```python
from build123d import *

# Parameters (mm, degrees)
SKETCH1_W                                           = 570
SKETCH1_H                                           = 160
BOSS_EXTRUDE1_DEPTH                                 = 12
SKETCH2_W                                           = 24
SKETCH2_H                                           = 246.506816481
SKETCH2_W_2                                         = 20
SKETCH2_H_2                                         = 260.473208351
CUT_EXTRUDE1_DEPTH                                  = 2
SKETCH3_W                                           = 431
SKETCH3_H                                           = 32
CUT_EXTRUDE2_DEPTH                                  = 2
SKETCH4_W                                           = 12
SKETCH4_H                                           = 67
CUT_EXTRUDE3_DEPTH                                  = 297.258333216
M5_TAPPED_HOLE1_D                                   = 4.2
FILLET1_R                                           = 5
FILLET2_R                                           = 5
CHAMFER1_SIZE                                       = 2
CBORE_FOR_M5_HEX_SOCKET_HEAD_CAP_SCREW1_D           = 5.5
CBORE_FOR_M5_HEX_SOCKET_HEAD_CAP_SCREW1_CBORE_D     = 10
CBORE_FOR_M5_HEX_SOCKET_HEAD_CAP_SCREW1_CBORE_DEPTH = 5.4
SKETCH13_R                                          = 8
CUT_EXTRUDE4_DEPTH                                  = 18
SKETCH14_R                                          = 2.5
CUT_EXTRUDE5_DEPTH                                  = 12
SKETCH15_R                                          = 8
CUT_EXTRUDE6_DEPTH                                  = 12


with BuildPart() as part:
    # Sketch1 → Boss-Extrude1 (new body)
    with BuildSketch(Plane.XY):
        Rectangle(SKETCH1_W, SKETCH1_H)
    extrude(amount=BOSS_EXTRUDE1_DEPTH)

    # Sketch2 → Cut-Extrude1 (cut)
    with BuildSketch(Plane.XY.offset(12)):
        with Locations((-200, -10.474793902)):
            Rectangle(SKETCH2_W, SKETCH2_H)
        with Locations((253, -9.078154715)):
            Rectangle(SKETCH2_W_2, SKETCH2_H_2)
    extrude(amount=-CUT_EXTRUDE1_DEPTH, mode=Mode.SUBTRACT)

    # Sketch3 → Cut-Extrude2 (cut)
    with BuildSketch(Plane.XY.offset(12)):
        with Locations((27.5, 64)):
            Rectangle(SKETCH3_W, SKETCH3_H)
        with Locations((27.5, -64)):
            Rectangle(SKETCH3_W, SKETCH3_H)
    extrude(amount=-CUT_EXTRUDE2_DEPTH, mode=Mode.SUBTRACT)

    # Sketch4 → Cut-Extrude3 (cut, through all)
    with BuildSketch(Plane.XY.offset(12)):
        with Locations((-279, 0)):
            Rectangle(SKETCH4_W, SKETCH4_H)
    extrude(amount=-CUT_EXTRUDE3_DEPTH, mode=Mode.SUBTRACT)

    # M5 Tapped Hole1 (through all)
    with Locations(Plane.XY.offset(10)):
        with Locations((227.5, -59), (107.5, -59), (-172.5, -59), (-52.5, -59), (-172.5, 59), (-52.5, 59), (107.5, 59), (227.5, 59)):
            Hole(M5_TAPPED_HOLE1_D / 2)

    # Fillet1
    fillet1_edges = [part.edges().sort_by_distance(p)[0] for p in [
        (-188, 48, 11),
        (243, 48, 11),
        (-188, -48, 11),
        (243, -48, 11),
    ]]
    fillet(fillet1_edges, radius=FILLET1_R)

    # Fillet2
    fillet2_edges = [part.edges().sort_by_distance(p)[0] for p in [
        (285, -80, 6),
        (-285, -80, 6),
        (-285, 80, 6),
        (285, 80, 6),
    ]]
    fillet(fillet2_edges, radius=FILLET2_R)

    # Chamfer1
    chamfer1_edges = [part.edges().sort_by_distance(p)[0] for p in [
        (-285, -33.5, 6),
        (-285, 33.5, 6),
    ]]
    chamfer(chamfer1_edges, length=CHAMFER1_SIZE)

    # CBORE for M5 Hex Socket Head Cap Screw1 (through all)
    with Locations(Plane.XY.offset(12)):
        with Locations((275, 67.5), (-275, -67.5), (-275, 67.5), (275, -67.5)):
            CounterBoreHole(CBORE_FOR_M5_HEX_SOCKET_HEAD_CAP_SCREW1_D / 2, CBORE_FOR_M5_HEX_SOCKET_HEAD_CAP_SCREW1_CBORE_D / 2, CBORE_FOR_M5_HEX_SOCKET_HEAD_CAP_SCREW1_CBORE_DEPTH)

    # Sketch13 → Cut-Extrude4 (cut)
    with BuildSketch(Plane.XY.offset(12)):
        with Locations((-242.5, 0)):
            Circle(SKETCH13_R)
    extrude(amount=-CUT_EXTRUDE4_DEPTH, mode=Mode.SUBTRACT)

    # Sketch14 → Cut-Extrude5 (cut)
    with BuildSketch(Plane(origin=(0, 0, 0), x_dir=(-1, 0, 0), z_dir=(0, 0, -1))):
        with Locations((218.93, -23.570000001)):
            Circle(SKETCH14_R)
        with Locations((266.07, -23.569995906)):
            Circle(SKETCH14_R)
        with Locations((266.069995906, 23.570004094)):
            Circle(SKETCH14_R)
        with Locations((218.929995906, 23.569999999)):
            Circle(SKETCH14_R)
    extrude(amount=-CUT_EXTRUDE5_DEPTH, mode=Mode.SUBTRACT)

    # Sketch15 → Cut-Extrude6 (cut)
    with BuildSketch(Plane.XY.offset(12)):
        with Locations((274, 0)):
            Circle(SKETCH15_R)
    extrude(amount=-CUT_EXTRUDE6_DEPTH, mode=Mode.SUBTRACT)


solid = part.part
```
Work out the finished part from the listing and answer in its coordinate system (mm). A direction names the side the tool comes from. Give positions to 0.01 mm unless a question says otherwise; leave off trailing zeros. Loops run counter-clockwise (first coordinate to the right, second up) from the corner with the lowest first, then second, coordinate; pieces in that order, holes last. Notation, with made-up numbers: (20.25, 34.5) -> (51.25, 34.5) arc R14 ccw to (51.25, 42.5) -> close; hole circle Ø6 at (-33, -11). An arc over 180 degrees is marked (long way). Put each result on its own line as item: value. Start each with the question number.
Item 1: Which of the six approach directions +Z, -Z, +X, -X, +Y, -Y give full straight-line access (tool end or side, diameter ignored) to faces 1 (the face through (264, 1, 12)), 2 (the face through (-273, 65, 6.6)), 3 (the face through (-278, 33.5, 6))?
Item 2: The part is cut by section C-C (x = 57). Give the vertices of the cut face in (y, z).
Item 3: The part is cut by section B-B (y = 0). Give the vertices of the cut face in (x, z), then the cut area to 3 significant figures.
Item 4: The part is cut by section A-A (z = 4.75). State how many separate pieces and enclosed holes the cut face has, then the cut area to 3 significant figures.
Item 5: Find the intervals of material crossed by L1, parallel to Y at x = 275, z = 3.5; L2, parallel to Z at x = 153, y = 58.5; L3, parallel to X at y = -60, z = 6.25, in increasing order. Write a range as [from, to].
Item 6: The mould has two halves that part along Y. Classify faces 4 (the face through (-4, -80, 6)), 5 (the face through (279.77, -66, 9.34)), 6 (the face through (-4, 80, 6)): released by +Y, released by -Y, zero draft, split by the parting line, or undercut.
Item 7: Each of these flat-tipped pins is pushed along its axis until it touches: P1, Ø3, axis at y = -25.5, z = 2.5, coming from the -X side; P2, Ø5, axis at x = -274, y = -69.5, coming from the +Z side; P3, Ø5.5, axis at x = -172.5, y = -59, coming from the +Z side. Where does it stop, or does it pass through?
Answers below:
1. face 1: +Z, +X, -X, +Y, -Y
1. face 2: +Z
1. face 3: +Z, -Z, -X
2. outline: (-80, 0) -> (80, 0) -> (80, 10) -> (48, 10) -> (48, 12) -> (-48, 12) -> (-48, 10) -> (-80, 10) -> close
3. outline: (-273, 0) -> (-250.5, 0) -> (-250.5, 12) -> (-273, 12) -> close; (-234.5, 0) -> (266, 0) -> (266, 12) -> (263, 12) -> (263, 10) -> (243, 10) -> (243, 12) -> (-188, 12) -> (-188, 10) -> (-212, 10) -> (-212, 12) -> (-234.5, 12) -> close; (282, 0) -> (285, 0) -> (285, 12) -> (282, 12) -> close
3. area: 6,220 mm2
4. separate pieces: 1
4. enclosed holes: 18
4. area: 89,700 mm2
5. L1: [-80, -70.25], [-64.75, -7.94], [7.94, 64.75], [70.25, 80]
5. L2: [0, 10]
5. L3: [-285, -174.35], [-170.65, -54.35], [-50.65, 105.65], [109.35, 225.65], [229.35, 285]
6. face 4: released by -Y
6. face 5: undercut
6. face 6: released by +Y
7. P1: x = -273
7. P2: z = 6.6
7. P3: z = 10
